Part model, mm, in its own coordinate system. Face numbers are marked on the shaded views. A direction names the side the tool comes from. Give positions to 0.01 mm unless a question says otherwise; leave off trailing zeros. Write each loop counter-clockwise with the first axis right and the second up, starting at its lowest first coordinate (ties: lowest second). Pieces come first, ordered by that corner, then holes. Notation, with made-up numbers: M 17,84.5 L 70,84.5 A18 ccw 70,109.5 Z; hole C 31.5,-38.75 d10. An arc over 180 degrees is marked long. Use a Markdown table: item, result.
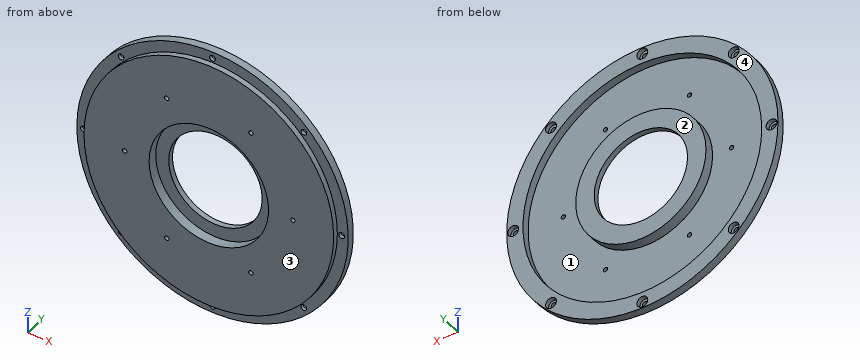
```python
from build123d import *

# Parameters (mm, degrees)
SKETCH2_R          = 2.65
CUT_EXTRUDE1_DEPTH = 10
SKETCH3_R          = 5
CUT_EXTRUDE3_DEPTH = 4
SKETCH4_R          = 2
CUT_EXTRUDE4_DEPTH = 20


with BuildPart() as part:
    # Sketch1 → Revolve1 (revolve)
    with BuildSketch(Plane.XY):
        Polygon((-125, 132), (-115, 132), (-115, 127), (-55, 127), (-55, 136), (-43, 136), (-43, 141), (-60, 141), (-60, 132), (-110, 132), (-110, 139), (-125, 139), align=None)
    revolve(axis=Axis((0, 0, 0), (0, -1, 0)))

    # Sketch2 → Cut-Extrude1 (cut)
    with BuildSketch(Plane(origin=(0, 139, 0), x_dir=(1, 0, 0), z_dir=(0, 1, 0))):
        with Locations(Location((0, 119, 0), (0, 0, 180))):
            Circle(SKETCH2_R)
        with Locations(Location((84.145706961, 84.145706961, 0), (0, 0, 180))):
            Circle(SKETCH2_R)
        with Locations(Location((119, 0, 0), (0, 0, 180))):
            Circle(SKETCH2_R)
        with Locations(Location((84.145706961, -84.145706961, 0), (0, 0, 180))):
            Circle(SKETCH2_R)
        with Locations(Location((0, -119, 0), (0, 0, 180))):
            Circle(SKETCH2_R)
        with Locations(Location((-84.145706961, -84.145706961, 0), (0, 0, 180))):
            Circle(SKETCH2_R)
        with Locations(Location((-119, 0, 0), (0, 0, 180))):
            Circle(SKETCH2_R)
        with Locations(Location((-84.145706961, 84.145706961, 0), (0, 0, 180))):
            Circle(SKETCH2_R)
    extrude(amount=-CUT_EXTRUDE1_DEPTH, mode=Mode.SUBTRACT)

    # Sketch3 → Cut-Extrude3 (cut)
    with BuildSketch(Plane(origin=(0, 139, 0), x_dir=(1, 0, 0), z_dir=(0, 1, 0))):
        with Locations(Location((0, 119, 0), (0, 0, 180))):
            Circle(SKETCH3_R)
        with Locations(Location((84.145706961, 84.145706961, 0), (0, 0, 180))):
            Circle(SKETCH3_R)
        with Locations(Location((119, 0, 0), (0, 0, 180))):
            Circle(SKETCH3_R)
        with Locations(Location((84.145706961, -84.145706961, 0), (0, 0, 180))):
            Circle(SKETCH3_R)
        with Locations(Location((0, -119, 0), (0, 0, 180))):
            Circle(SKETCH3_R)
        with Locations(Location((-84.145706961, -84.145706961, 0), (0, 0, 180))):
            Circle(SKETCH3_R)
        with Locations(Location((-119, 0, 0), (0, 0, 180))):
            Circle(SKETCH3_R)
        with Locations(Location((-84.145706961, 84.145706961, 0), (0, 0, 180))):
            Circle(SKETCH3_R)
    extrude(amount=-CUT_EXTRUDE3_DEPTH, mode=Mode.SUBTRACT)

    # Sketch4 → Cut-Extrude4 (cut)
    with BuildSketch(Plane(origin=(0, 132, 0), x_dir=(1, 0, 0), z_dir=(0, 1, 0))):
        with Locations(Location((77.5, 0, 0), (0, 0, 180))):
            Circle(SKETCH4_R)
        with Locations(Location((38.75, -67.116968793, 0), (0, 0, 180))):
            Circle(SKETCH4_R)
        with Locations(Location((-38.75, -67.116968793, 0), (0, 0, 180))):
            Circle(SKETCH4_R)
        with Locations(Location((-77.5, 0, 0), (0, 0, 180))):
            Circle(SKETCH4_R)
        with Locations(Location((-38.75, 67.116968793, 0), (0, 0, 180))):
            Circle(SKETCH4_R)
        with Locations(Location((38.75, 67.116968793, 0), (0, 0, 180))):
            Circle(SKETCH4_R)
    extrude(amount=-CUT_EXTRUDE4_DEPTH, mode=Mode.SUBTRACT)


solid = part.part
```
1. Drill centre lines: L1, parallel to Z at x = 0, y = 137.95; L2, parallel to X at y = 138, z = -44; L3, parallel to X at y = 134.75, z = 4. Where is each one in solid material? Low to high.
Findings below:
| item | result |
|---|---|
| L1 | -125 to -124, -114 to -110, -60 to -43, 43 to 60, 110 to 114, 124 to 125 |
| L2 | -117 to -100.82, -40.79 to 40.79, 100.82 to 117 |
| L3 | -124.94 to -109.93, -59.87 to -54.85, 54.85 to 59.87, 109.93 to 124.94 |
2. Cut at C-C, the plane x = 95.5. Give the cut face in (y, z).
Findings below:
| item | result |
|---|---|
| outline | M 127,-64.07 L 132,-64.07 L 132,-80.65 L 139,-80.65 L 139,-54.59 L 132,-54.59 L 132,54.59 L 139,54.59 L 139,80.65 L 132,80.65 L 132,64.07 L 127,64.07 Z |
3. Two-plate mould, pull along Z, no slides. Class the marked faces 1 and 2: released by +Z, released by -Z, zero draft, split by the parting line, or undercut.
Findings below:
| item | result |
|---|---|
| face 1 | undercut |
| face 2 | zero draft |
4. Drop flat-ended pins along their axis: P1, Ø11.5, axis at x = -119, z = 0, coming from the +Y side; P2, Ø2, axis at x = -82.5, y = 132, coming from the -Z side; P3, Ø2, axis at x = 99.5, y = 138, coming from the +Z side; P4, Ø4, axis at x = 84.15, z = 84.15, coming from the +Y side. Give the stop position or say it passes through.
Findings below:
| item | result |
|---|---|
| P1 | y = 139 |
| P2 | z = -94.78 |
| P3 | z = 76.96 |
| P4 | through |
5. Cut at A-A, the plane z = 30. Give the cut face in (x, y).
Findings below:
| item | result |
|---|---|
| outline | M -121.35,132 L -111.02,132 L -111.02,127 L -46.1,127 L -46.1,136 L -30.81,136 L -30.81,141 L -51.96,141 L -51.96,132 L -105.83,132 L -105.83,139 L -121.35,139 Z; M 30.81,136 L 46.1,136 L 46.1,127 L 111.02,127 L 111.02,132 L 121.35,132 L 121.35,139 L 105.83,139 L 105.83,132 L 51.96,132 L 51.96,141 L 30.81,141 Z |
6. Tool access for the marked faces 3 and 4: list every direction of +Z, -Z, +X, -X, +Y, -Y with a clear straight run to the whole face (end or side of a thin tool).
Findings below:
| item | result |
|---|---|
| face 3 | +Z, -Z, +X, -X, -Y |
| face 4 | +Y |
7. Cut at B-B, the plane x = -19.5. Give the cut face in (y, z), then the cut area to 3 significant figures.
Findings below:
| item | result |
|---|---|
| outline | M 127,-113.33 L 132,-113.33 L 132,-123.47 L 139,-123.47 L 139,-108.26 L 132,-108.26 L 132,-56.74 L 141,-56.74 L 141,-38.32 L 136,-38.32 L 136,-51.43 L 127,-51.43 Z; M 127,51.43 L 136,51.43 L 136,38.32 L 141,38.32 L 141,56.74 L 132,56.74 L 132,108.26 L 139,108.26 L 139,123.47 L 132,123.47 L 132,113.33 L 127,113.33 Z |
| area | 1,060 mm2 |
